from build123d import *

# Parameters (mm, degrees)
BASE_PLATE_14MM_DEPTH        = 7
SIDE_PLATE_14MM_DEPTH        = 14
SLOTTED_END_PLATE_PROFILE_R  = 10
SLOTTED_END_PLATE_14MM_DEPTH = 14


with BuildPart() as part:
    # Base Plate Profile → Base Plate 14mm (new, symmetric)
    with BuildSketch(Plane.XY):
        with BuildLine():
            Line((0, 0), (0, 75))
            Line((0, 75), (32, 75))
            ThreePointArc((32, 75), (51.798989873, 66.798989873), (60, 47))
            Line((60, 47), (60, 0))
            Line((60, 0), (40, 0))
            Line((40, 0), (40, 28))
            Line((40, 28), (20, 28))
            Line((20, 28), (20, 0))
            Line((20, 0), (0, 0))
        make_face()
    extrude(amount=BASE_PLATE_14MM_DEPTH, both=True)

    # Side Plate Profile → Side Plate 14mm (add)
    with BuildSketch(Plane.ZY):
        with BuildLine():
            Line((-7, 75), (82, 75))
            Line((82, 75), (82, 58))
            ThreePointArc((82, 58), (42.329041508, 40.541426156), (27, 0))
            Line((27, 0), (7, 0))
            Line((7, 0), (-7, 0))
            Line((-7, 0), (-7, 75))
        make_face()
    extrude(amount=SIDE_PLATE_14MM_DEPTH)

    # Slotted End Plate Profile → Slotted End Plate 14mm (add)
    with BuildSketch(Plane(origin=(0, 75, 0), x_dir=(1, 0, 0), z_dir=(0, 1, 0))):
        with BuildLine():
            Line((-53.037054902, -79.973094831), (-14, -82))
            Line((-14, -82), (-14, 7))
            Line((-14, 7), (-66.238116475, -45.954501104))
            ThreePointArc((-66.238116475, -45.954501104), (-70.645345128, -67.23540635), (-53.037054902, -79.973094831))
        make_face()
        with Locations(Location((-52, -60, 0), (0, 0, 270))):
            Circle(SLOTTED_END_PLATE_PROFILE_R, mode=Mode.SUBTRACT)
    extrude(amount=-SLOTTED_END_PLATE_14MM_DEPTH)


solid = part.part
Read the model definition and answer for the solid it produces. Units are mm, in the model's axes. A direction names the side the tool comes from. Give positions to 0.01 mm unless a question says otherwise; leave off trailing zeros. Write each loop counter-clockwise with the first axis right and the second up, starting at its lowest first coordinate (ties: lowest second). Pieces come first, ordered by that corner, then holes. Notation, with made-up numbers: (-40, 11.25) - (-30, 11.25) arc R29 ccw to (-30, 47.25) - close; hole circle Ø5 at (86, 56). An arc over 180 degrees is marked (long way). Use CSV: the item, a comma, the result in double quotes. Start each with the question number.
Item 1: The part is cut by section A-A, the plane y = 9. Give the vertices of the cut face in (x, z).
Item 2: The mould has two halves that part along X. Classify faces 1 (the cylindrical face through (-6.9, 40.99, 42.76)), 2 (the flat face through (20, 14, 0)), 3 (the flat face through (60, 24, 0)): pulls with the +X half, pulls with the -X half, needs draft (parallel to the pull), parting line crosses it, or undercut.
Item 3: Consider line 1 (X direction, y = 71, z = 60); line 2 (X direction, y = 15.5, z = 13); line 3 (Y direction, x = -65, z = 52.5). Determine where each line is inside the solid, lowest interval first.
Item 4: The part is cut by section C-C, the plane x = -10. Give the vertices of the cut face in (y, z).
Item 5: The part is cut by section D-D, the plane z = 47.5. Give the vertices of the cut face in (x, y), and give its area (3 significant figures).
Item 6: For faces 4 (the flat face through (-14, 38, 18)), 5 (the flat face through (30, 28, 0)), 6 (the flat face through (30, 38, 7)), determine the directions among +Z, -Z, +X, -X, +Y, -Y from which every point of the face is accessible in a straight line to the end or side of a thin tool.
Item 7: Flat-ended cylindrical pins translate along their axes: P1, Ø10, axis at x = 1.5, z = 26, coming from the -Y side; P2, Ø17.5, axis at x = -32.5, z = 57, coming from the -Y side; P3, Ø11, axis at y = 16.5, z = -2, coming from the -X side; P4, Ø4, axis at x = 32, z = 3, coming from the -Y side. Find the tip coordinate at first contact, or state that the pin passes through.
Item 8: The part is cut by section B-B, the plane z = 60. Give the vertices of the cut face in (x, y).
Taken from the geometry:
1,outline,"(-14, -7) - (20, -7) - (20, 7) - (0, 7) - (0, 27.4) - (-14, 27.4) - close; (40, -7) - (60, -7) - (60, 7) - (40, 7) - close"
2,face 1,"needs draft"
2,face 2,"undercut"
2,face 3,"pulls with the +X half"
3,line 1,"-72 to -62, -42 to 0"
3,line 2,"-14 to 0"
3,line 3,"61 to 75"
4,outline,"(0, -7) - (75, -7) - (75, 82) - (58, 82) arc R56 cw to (0, 27) - close"
5,outline,"(-67.61, 61) - (-14, 61) - (-14, 45.35) - (0, 45.35) - (0, 75) - (-67.61, 75) - close"
5,area,"1,170 mm2"
6,face 4,"+Z, -Z, -X, -Y"
6,face 5,"+Z, -Z, -Y"
6,face 6,"+Z, +X, +Y, -Y"
7,P1,"y = 0"
7,P2,"y = 61"
7,P3,"x = -14"
7,P4,"y = 28"
8,outline,"(-72, 61) - (-62, 61) - (-62, 75) - (-72, 75) - close; (-42, 61) - (-14, 61) - (-14, 53.08) - (0, 53.08) - (0, 75) - (-42, 75) - close"
